from build123d import *

# Parameters (mm, degrees)
GB_6728_1986_RECTANGULAR_HOLLOW_SECTION_DEPTH = 53
CUT_EXTRUDE1_DEPTH                            = 101.04498988
CUT_EXTRUDE1_DEPTH_BACK                       = 101.04498988


with BuildPart() as part:
    # Sketch1 → GB/6728-1986 rectangular hollow section 120 X 60 X 4(1) (new body)
    with BuildSketch(Plane.YZ):
        with BuildLine():
            Line((-22, -60), (22, -60))
            ThreePointArc((22, -60), (27.656854249, -57.656854249), (30, -52))
            Line((30, -52), (30, 52))
            ThreePointArc((30, 52), (27.656854249, 57.656854249), (22, 60))
            Line((22, 60), (-22, 60))
            ThreePointArc((-22, 60), (-27.656854249, 57.656854249), (-30, 52))
            Line((-30, 52), (-30, -52))
            ThreePointArc((-30, -52), (-27.656854249, -57.656854249), (-22, -60))
        make_face()
        with BuildLine():
            Line((-22, -56), (22, -56))
            ThreePointArc((22, -56), (24.828427125, -54.828427125), (26, -52))
            Line((26, -52), (26, 52))
            ThreePointArc((26, 52), (24.828427125, 54.828427125), (22, 56))
            Line((22, 56), (-22, 56))
            ThreePointArc((-22, 56), (-24.828427125, 54.828427125), (-26, 52))
            Line((-26, 52), (-26, -52))
            ThreePointArc((-26, -52), (-24.828427125, -54.828427125), (-22, -56))
        make_face(mode=Mode.SUBTRACT)
    extrude(amount=GB_6728_1986_RECTANGULAR_HOLLOW_SECTION_DEPTH)

    # Sketch3 → Cut-Extrude1 (cut, two sides: drawn at the far end of the back side and taken through both)
    with BuildSketch(Plane.XZ.offset(30).offset(-CUT_EXTRUDE1_DEPTH_BACK)):
        Polygon((53, 60), (50, -60), (53, -60), align=None)
    extrude(amount=CUT_EXTRUDE1_DEPTH + CUT_EXTRUDE1_DEPTH_BACK, mode=Mode.SUBTRACT)


solid = part.part
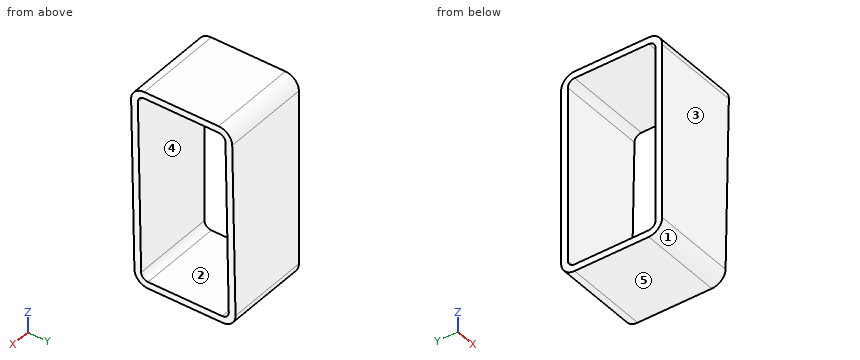
The model under review builds one solid part; all positions refer to its coordinate system, in mm. Face numbers are marked on the shaded views. A direction names the side the tool comes from. Round coordinates to 2 decimals unless told otherwise and drop trailing zeros. Order: outer loops, then holes, each group sorted by start corner. A loop starts at its lowest first (then second) coordinate and runs counter-clockwise, first axis right, second up. Notation, with made-up numbers: (49, 68.5) -> (71, 68.5) arc R20 cw to (71, 101.5) -> close; hole circle Ø6 at (-2.5, 63.25). An arc over 180 degrees is marked (long way). Write item = value, one per line. Start each with the question number.
Item 1: Clearance check with flat-ended pins moving along their axes: pin 1 Ø5 at (x, y) = (23.5, -23) entering from -Z; pin 2 Ø12 at (y, z) = (-16, -14.5) entering from +X. State where each tip first meets the part, or that it passes through.
Item 2: Consider section A-A on z = -12. Write out the cut boundary in (x, y), plus the area to 3 significant figures.
Item 3: Consider section C-C on x = 8. Write out the cut boundary in (y, z).
Item 4: For line 1 along Y through (x, z) = (45, 34); line 2 along Z through (x, y) = (7, 11); line 3 along Z through (x, y) = (13, -23.5), list the stretches that pass through material, from the lowest coordinate up.
Item 5: Mouldability with a two-part tool opening along Y and no side actions: class the marked faces 3, 4 and 5 as released by +Y, released by -Y, zero draft, split by the parting line, or undercut.
Item 6: For the marked faces 1 and 2, list the 3-axis set-ups (+Z, -Z, +X, -X, +Y, -Y) from which the entire face can be reached by the end or side of a thin tool; tool diameter is ignored.
Item 7: Consider section B-B on y = -6.5. Write out the cut boundary in (x, z).
Conclusion:
q1.pin_1 = -60
q1.pin_2 = through
q2.outline = (0, -30) -> (51.2, -30) -> (51.2, -26) -> (0, -26) -> close; (0, 26) -> (51.2, 26) -> (51.2, 30) -> (0, 30) -> close
q2.area = 410 mm2
q3.outline = (-30, -52) arc R8 ccw to (-22, -60) -> (22, -60) arc R8 ccw to (30, -52) -> (30, 52) arc R8 ccw to (22, 60) -> (-22, 60) arc R8 ccw to (-30, 52) -> close; hole (-26, -52) arc R4 ccw to (-22, -56) -> (22, -56) arc R4 ccw to (26, -52) -> (26, 52) arc R4 ccw to (22, 56) -> (-22, 56) arc R4 ccw to (-26, 52) -> close
q4.line_1 = -30 to -26, 26 to 30
q4.line_2 = -60 to -56, 56 to 60
q4.line_3 = -59.86 to -55.71, 55.71 to 59.86
q5.face_3 = released by -Y
q5.face_4 = undercut
q5.face_5 = zero draft
q6.face_1 = -Z, +X, -X, -Y
q6.face_2 = +X, -X
q7.outline = (0, -60) -> (50, -60) -> (50.1, -56) -> (0, -56) -> close; (0, 56) -> (52.9, 56) -> (53, 60) -> (0, 60) -> close
